from build123d import *

# Parameters (mm, degrees)
SKETCH1_W             = 240
SKETCH1_H             = 40
EXTRUDE1_DEPTH        = 6
M6_TAPPED_HOLE1_D     = 5
M6_TAPPED_HOLE1_DEPTH = 15
M6_TAPPED_HOLE1_TIP   = 1.502151548
CHAMFER1_SIZE         = 5


with BuildPart() as part:
    # Sketch1 → Extrude1 (new, symmetric)
    with BuildSketch(Plane(origin=(0, 0, 0), x_dir=(1, 0, 0), z_dir=(0, 1, 0))):
        Rectangle(SKETCH1_W, SKETCH1_H)
    extrude(amount=EXTRUDE1_DEPTH, both=True)

    # M6 Tapped Hole1
    with Locations(Plane(origin=(0, 6, 0), x_dir=(-1, 0, 0), z_dir=(0, 1, 0))):
        with Locations((100, 0), (0, 0), (-100, 0)):
            Hole(M6_TAPPED_HOLE1_D / 2, depth=M6_TAPPED_HOLE1_DEPTH)
            with Locations((0, 0, -(M6_TAPPED_HOLE1_DEPTH + M6_TAPPED_HOLE1_TIP / 2))):  # 118° drill point
                Cone(0, M6_TAPPED_HOLE1_D / 2, M6_TAPPED_HOLE1_TIP, mode=Mode.SUBTRACT)

    # Chamfer1
    chamfer1_edges = [part.edges().sort_by_distance(p)[0] for p in [
        (-120, 0, -20),
        (120, 0, -20),
        (120, 0, 20),
        (-120, 0, 20),
    ]]
    chamfer(chamfer1_edges, length=CHAMFER1_SIZE)


solid = part.part
Could you check a few things on this model? Use its own coordinates, in mm. Give positions to 0.01 mm unless a question says otherwise; leave off trailing zeros. Loops run counter-clockwise (first coordinate to the right, second up) from the corner with the lowest first, then second, coordinate; pieces in that order, holes last. Notation, with made-up numbers: (-21, 53) -> (11, 53) arc R31 ccw to (11, 83) -> close; hole circle Ø7 at (-16.75, 70.5). An arc over 180 degrees is marked (long way). Return JSON: item names as keys, results as strings.
Item 1: If we section it at B-B on z = -17: List the corners of the cut face in (x, y) for me, plus the area to 3 significant figures.
Geometry results:
{"outline": "(-118, -6) -> (118, -6) -> (118, 6) -> (-118, 6) -> close", "area": "2,830 mm²"}
Item 2: I need wall thicknesses on L1, parallel to Z at x = -100, y = 2.25; L2, parallel to X at y = 0, z = -1. Which ranges of each line are inside material? Lowest first, please. Write a range as from..to.
Geometry results:
{"L1": "z = -20..-2.5, 2.5..20", "L2": "x = -120..-102.29, -97.71..-2.29, 2.29..97.71, 102.29..120"}
Item 3: I'm going to push a flat-ended pin straight in: pin 1 (4.5 mm diameter, centred on x = 0, z = 0, fed in from +Y). Where does the tip first touch, or does it pass through?
Geometry results:
{"pin 1": "passes through"}
Item 4: If we section it at A-A on x = -100: List the corners of the cut face in (y, z) for me.
Geometry results:
{"outline": "(-6, -20) -> (6, -20) -> (6, -2.5) -> (-6, -2.5) -> close; (-6, 2.5) -> (6, 2.5) -> (6, 20) -> (-6, 20) -> close"}
Item 5: We'd pull the mould along Z, two halves only. Please class faces 1 (the flat face through (-2, 6, -5)), 2 (the flat face through (-117, 0, -18)), 3 (the cylindrical face through (-97.615, -0.084, 0.751)): +Z half, -Z half, draft (parallel to the pull), parting line (faces both ways), or undercut.
Geometry results:
{"face 1": "draft", "face 2": "-Z half", "face 3": "undercut"}
